For this review, take the finished solid that the model builds, in its own axes (mm). Face numbers are marked on the shaded views. A direction names the side the tool comes from. Coordinates: 2 decimals unless noted, no trailing zeros. Loops run counter-clockwise (first coordinate to the right, second up) from the corner with the lowest first, then second, coordinate; pieces in that order, holes last. Notation, with made-up numbers: (-32.75, 67) -> (25.25, 67) arc R20 ccw to (25.25, 78) -> close; hole circle Ø10 at (85.25, 73). An arc over 180 degrees is marked (long way). Answer in a Markdown table with one row per item.
from build123d import *

# Parameters (mm, degrees)
CUT_EXTRUDE1_DEPTH = 6
FILLET1_R          = 0.4
CHAMFER1_SIZE      = 1


with BuildPart() as part:
    # Sketch1 → Base-Revolve (revolve)
    with BuildSketch(Plane.XY, mode=Mode.PRIVATE) as base_revolve_sk:
        with BuildLine():
            Line((0, 0), (0, 8))
            Line((0, 8), (10, 8))
            Line((10, 8), (10, 5.6))
            ThreePointArc((10, 5.6), (10.026649761, 5.456439562), (10.103047997, 5.332008381))
            Line((10.103047997, 5.332008381), (10.723047997, 4.645008381))
            ThreePointArc((10.723047997, 4.645008381), (10.857514074, 4.547488955), (11.02, 4.513))
            Line((11.02, 4.513), (14.5, 4.513))
            Line((14.5, 4.513), (14.987, 5))
            Line((14.987, 5), (40, 5))
            Line((40, 5), (40, 0))
            Line((40, 0), (0, 0))
        make_face()
    revolve(base_revolve_sk.sketch.rotate(Axis((0, 0, 0), (-1, 0, 0)), 90), axis=Axis((0, 0, 0), (-1, 0, 0)))

    # Sketch2 → Cut-Extrude1 (cut)
    with BuildSketch(Plane.ZY):
        Polygon((3.962066222, -2.2875), (3.962066222, 2.2875), (0, 4.575), (-3.962066222, 2.2875), (-3.962066222, -2.2875), (0, -4.575), align=None)
    extrude(amount=-CUT_EXTRUDE1_DEPTH, mode=Mode.SUBTRACT)

    # Sketch13 → Cut-Revolve4 (revolve, cut)
    with BuildSketch(Plane.XY):
        Polygon((0, 4.575), (0.612933778, 3.962066222), (0, 3.962066222), align=None)
    revolve(axis=Axis((0, 0, 0), (-1, 0, 0)), mode=Mode.SUBTRACT)

    # Sketch16 → Cut-Revolve5 (revolve, cut)
    with BuildSketch(Plane.XY, mode=Mode.PRIVATE) as cut_revolve5_sk:
        Polygon((8.641377482, 0), (6, 4.575), (6, 0), align=None)
    revolve(cut_revolve5_sk.sketch.rotate(Axis((6, 0, 0), (1, 0, 0)), 180), axis=Axis((6, 0, 0), (1, 0, 0)), mode=Mode.SUBTRACT)

    # Fillet1
    fillet1_edges = [part.edges().sort_by_distance(p)[0] for p in [
        (0, 0, 8),
    ]]
    fillet(fillet1_edges, radius=FILLET1_R)

    # Chamfer1
    chamfer1_edges = [part.edges().sort_by_distance(p)[0] for p in [
        (40, 0, 5),
    ]]
    chamfer(chamfer1_edges, length=CHAMFER1_SIZE)


solid = part.part
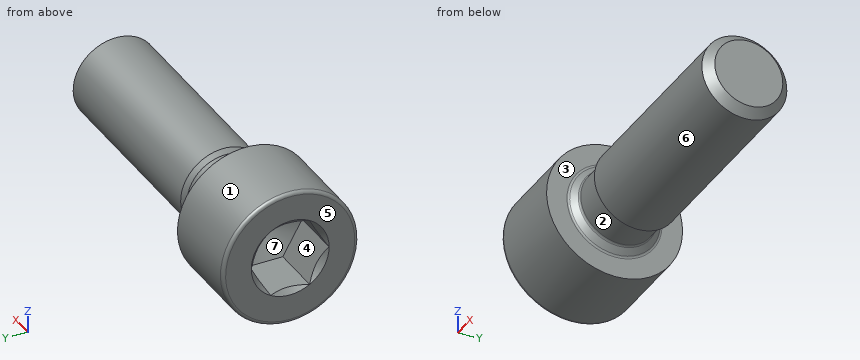
Item 1: For the marked faces 1, 2, 3 and 4, list the 3-axis set-ups (+Z, -Z, +X, -X, +Y, -Y) from which the entire face can be reached by the end or side of a thin tool; tool diameter is ignored.
Worked answers:
| item | result |
|---|---|
| face 1 | +X, -X |
| face 2 | none |
| face 3 | +X |
| face 4 | -X |
Item 2: Insertion check: pin 1 (1 mm diameter, centred on x = 14, z = 5.5, fed in from -Y); pin 2 (1 mm diameter, centred on x = 21, z = 4.5, fed in from +Y); pin 3 (3 mm diameter, centred on x = 10, y = -3.5, fed in from +Z); pin 4 (1.5 mm diameter, centred on x = 33, z = -2.5, fed in from -Y). Each pin has a flat end and moves straight along its axis. Give the tip position at first contact, or say it passes through.
Worked answers:
| item | result |
|---|---|
| pin 1 | through |
| pin 2 | y = 3 |
| pin 3 | z = 7.75 |
| pin 4 | y = -4.68 |
Item 3: The part is to be moulded in two halves that separate along Y. For the marked faces 5, 6 and 7, say which applies: +Y half, -Y half, draft (parallel to the pull), parting line (faces both ways), or undercut.
Worked answers:
| item | result |
|---|---|
| face 5 | draft |
| face 6 | parting line |
| face 7 | undercut |
Item 4: For L1, parallel to Y at x = 15.5, z = 3; L2, parallel to X at y = 1, z = -6.25; L3, parallel to X at y = 2, z = -4.25, list the stretches that pass through material, from the lowest coordinate up.
Worked answers:
| item | result |
|---|---|
| L1 | -4 to 4 |
| L2 | 0 to 10 |
| L3 | 0 to 10.68, 14.68 to 39.3 |
Item 5: Take a section at A-A, the plane x = 29.5. State the section outline as (y, z) points.
Worked answers:
| item | result |
|---|---|
| outline | circle Ø10 at (0, 0) |
